Input: dimensioned drawing with shaded views. Units: mm. Origin: part minimum x, y, z. Round coordinates to 2 decimals unless told otherwise and drop trailing zeros. Loops run counter-clockwise (first coordinate to the right, second up) from the corner with the lowest first, then second, coordinate; pieces in that order, holes last. Notation, with made-up numbers: (47, 6) - (83, 6) arc R27 ccw to (83, 24) - close; hole circle Ø11 at (61, -1). An arc over 180 degrees is marked (long way). One line per question, with ' | ' between items.
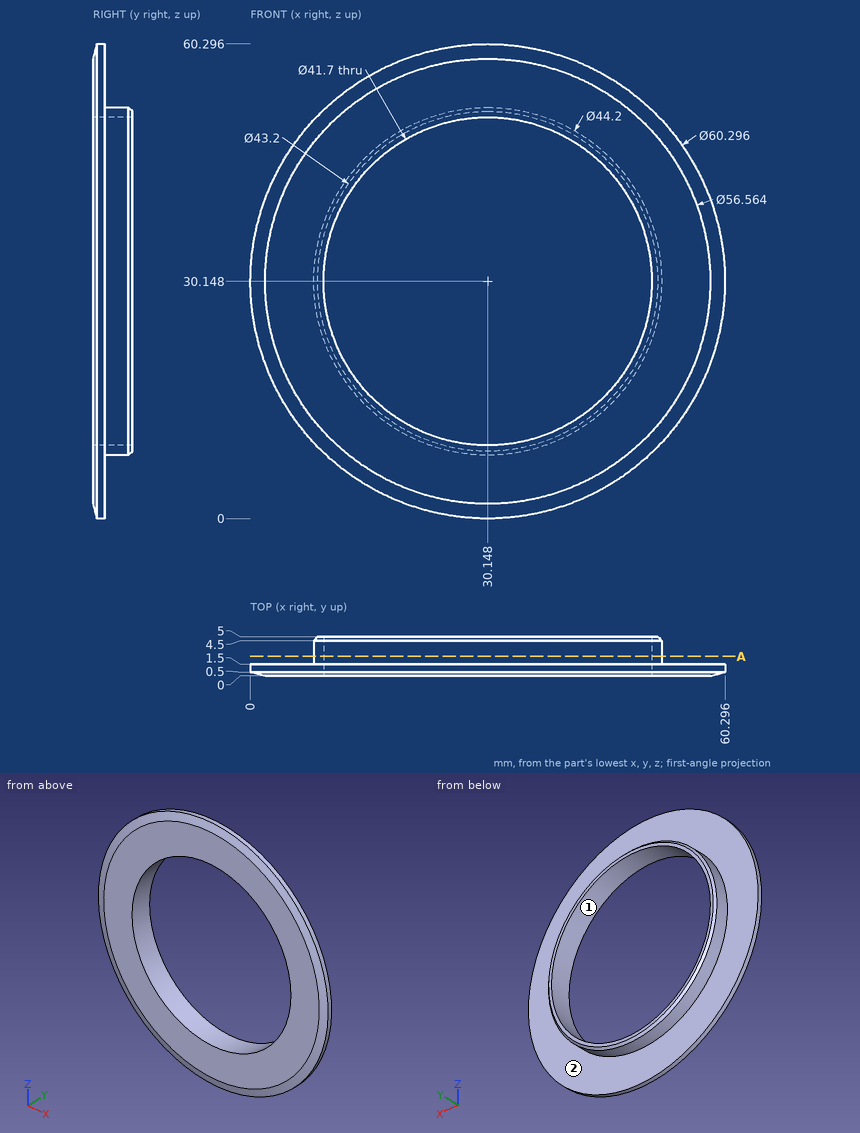
1. Mould query, pull axis Z, two halves, no side actions, for the marked faces 1 and 2. Classes: released by +Z, released by -Z, zero draft, split by the parting line, or undercut.
Worked out:
face 1: undercut | face 2: zero draft
2. Section query A-A, the plane y = 2.5. Return loops of the section in (x, z), plus the area to 3 significant figures.
Worked out:
outline: circle Ø44.2 at (30.15, 30.15); hole circle Ø41.7 at (30.15, 30.15) | area: 169 mm2
3. Material intervals for probe 1 along X at (y, z) = (1.65, 29.5); probe 2 along X at (y, z) = (3.4, 33.5); probe 3 along Y at (x, z) = (9.5, 18.5), sorted ascending.
Worked out:
probe 1: x = 8.06 to 9.31, 50.99 to 52.24 | probe 2: x = 8.3 to 9.57, 50.73 to 51.99 | probe 3: y = 0 to 1.5
